Input: part model. Units: mm. Frame: model coordinates. A direction names the side the tool comes from. Give positions to 0.01 mm unless a question says otherwise; leave off trailing zeros. Write each loop counter-clockwise with the first axis right and the second up, starting at its lowest first coordinate (ties: lowest second). Pieces come first, ordered by that corner, then holes. Notation, with made-up numbers: M 80,29 L 100,29 A24 cw 100,54 Z; hole C 26,81.5 d10. An arc over 180 degrees is marked long. Use CSV: the item, a comma, the result in double quotes. Start each with the question number.
from build123d import *

# Parameters (mm, degrees)
SKETCH1_R           = 5
BOSS_EXTRUDE1_DEPTH = 10
SKETCH2_W           = 7
SKETCH2_H           = 7.141428428
BOSS_EXTRUDE2_DEPTH = 20
FILLET1_R           = 1
SKETCH3_W           = 5
SKETCH3_H           = 5
BOSS_EXTRUDE3_DEPTH = 20
FILLET2_R           = 0.5
BOSS_EXTRUDE4_DEPTH = 8


with BuildPart() as part:
    # Sketch1 → Boss-Extrude1 (new body)
    with BuildSketch(Plane.XY):
        Circle(SKETCH1_R)
    extrude(amount=BOSS_EXTRUDE1_DEPTH)

    # Sketch2 → Boss-Extrude2 (add)
    with BuildSketch(Plane.XY.offset(10)):
        Rectangle(SKETCH2_W, SKETCH2_H)
    extrude(amount=BOSS_EXTRUDE2_DEPTH)

    # Fillet1
    fillet1_edges = [part.edges().sort_by_distance(p)[0] for p in [
        (3.5, -3.570714214, 20),
        (3.5, 3.570714214, 20),
        (-3.5, 3.570714214, 20),
        (-3.5, -3.570714214, 20),
    ]]
    fillet(fillet1_edges, radius=FILLET1_R)

    # Sketch3 → Boss-Extrude3 (add)
    with BuildSketch(Plane.XY.offset(30)):
        Rectangle(SKETCH3_W, SKETCH3_H)
    extrude(amount=BOSS_EXTRUDE3_DEPTH)

    # Fillet2
    fillet2_edges = [part.edges().sort_by_distance(p)[0] for p in [
        (-2.5, 2.5, 40),
        (-2.5, -2.5, 40),
        (2.5, -2.5, 40),
        (2.5, 2.5, 40),
    ]]
    fillet(fillet2_edges, radius=FILLET2_R)

    # Sketch4 → Boss-Extrude4 (add)
    with BuildSketch(Plane.XY.offset(50)):
        Polygon((1, 1.732050808), (-1, 1.732050808), (-2, 0), (-1, -1.732050808), (1, -1.732050808), (2, 0), align=None)
    extrude(amount=BOSS_EXTRUDE4_DEPTH)


solid = part.part
Q1. Set-up query: faces 1 (the flat face through (-1.49, 0.88, 53.94)), 2 (the flat face through (2.5, 0, 40)), 3 (the flat face through (-3.5, 0, 20)). Return all of +Z, -Z, +X, -X, +Y, -Y with unobstructed straight access to the full face (end or side cutting, diameter ignored); none if empty.
Q2. Material intervals for L1, parallel to Z at x = -3, y = -2; L2, parallel to Y at x = 2.5, z = 19.5; L3, parallel to X at y = 1, z = 49, sorted ascending. Write a range as [from, to].
Q3. Section B-B, the plane x = 0. Return the cut outline in (y, z), and give its area (3 significant figures).
Q4. Section D-D, the plane z = 42. Return the cut outline in (x, y), and give its area (3 significant figures).
Q5. First-contact query: pin 1 Ø2 at (x, z) = (-1, 44.5) entering from +Y; pin 2 Ø2.5 at (x, z) = (-1, 20.5) entering from +Y; pin 3 Ø3 at (x, z) = (-0.5, 18.5) entering from -Y. Flat tips, straight axial feed; report the tip coordinate or a pass-through.
Q6. Section C-C, the plane y = -0.5. Return the cut outline in (x, z), and give its area (3 significant figures).
Q7. Section A-A, the plane z = 16. Return the cut outline in (x, y), and give its area (3 significant figures).
Check result:
1,face 1,"+Z, -X, +Y"
1,face 2,"+Z, +X, +Y, -Y"
1,face 3,"+Z, -X, +Y, -Y"
2,L1,"z = [0, 30]"
2,L2,"y = [-3.57, 3.57]"
2,L3,"x = [-2.5, 2.5]"
3,outline,"M -5,0 L 5,0 L 5,10 L 3.57,10 L 3.57,30 L 2.5,30 L 2.5,50 L 1.73,50 L 1.73,58 L -1.73,58 L -1.73,50 L -2.5,50 L -2.5,30 L -3.57,30 L -3.57,10 L -5,10 Z"
3,area,"371 mm²"
4,outline,"M -2.5,-2 A0.5 ccw -2,-2.5 L 2,-2.5 A0.5 ccw 2.5,-2 L 2.5,2 A0.5 ccw 2,2.5 L -2,2.5 A0.5 ccw -2.5,2 Z"
4,area,"24.8 mm²"
5,pin 1,"stops at y = 2.5"
5,pin 2,"stops at y = 3.57"
5,pin 3,"stops at y = -3.57"
6,outline,"M -4.97,0 L 4.97,0 L 4.97,10 L 3.5,10 L 3.5,30 L 2.5,30 L 2.5,50 L 1.71,50 L 1.71,58 L -1.71,58 L -1.71,50 L -2.5,50 L -2.5,30 L -3.5,30 L -3.5,10 L -4.97,10 Z"
6,area,"367 mm²"
7,outline,"M -3.5,-2.57 A1 ccw -2.5,-3.57 L 2.5,-3.57 A1 ccw 3.5,-2.57 L 3.5,2.57 A1 ccw 2.5,3.57 L -2.5,3.57 A1 ccw -3.5,2.57 Z"
7,area,"49.1 mm²"
